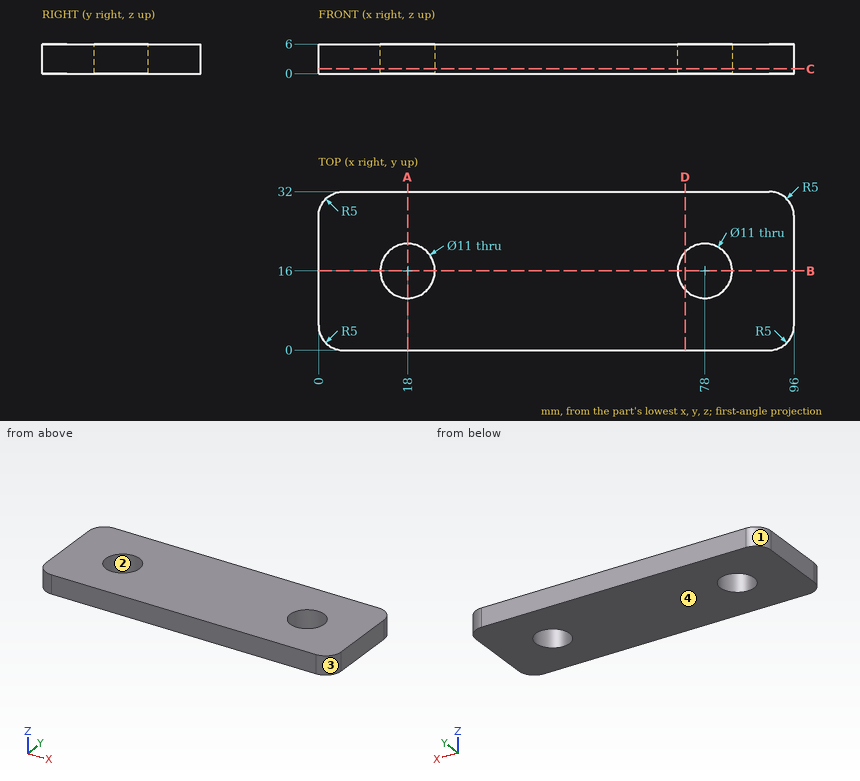
The drawing under review shows one solid part. Ordinate dimensions are in mm from its lowest x, y, z. Round coordinates to 2 decimals unless told otherwise and drop trailing zeros. Order: outer loops, then holes, each group sorted by start corner. A loop starts at its lowest first (then second) coordinate and runs counter-clockwise, first axis right, second up. Notation, with made-up numbers: (61, 83) -> (114, 83) arc R13 ccw to (114, 97) -> close; hole circle Ø1 at (21, -4). An arc over 180 degrees is marked (long way). Use a Markdown table: item, result.
Item 1: For pin 1 (10 mm diameter, centred on x = 78, y = 16, fed in from -Z), flat-tipped, find the tip position at first contact; note if it passes through.
Resolved:
| item | result |
|---|---|
| pin 1 | passes through |
Item 2: Take a section at C-C (z = 1). State the section outline as (x, y) points, plus the area to 3 significant figures.
Resolved:
| item | result |
|---|---|
| outline | (0, 5) arc R5 ccw to (5, 0) -> (91, 0) arc R5 ccw to (96, 5) -> (96, 27) arc R5 ccw to (91, 32) -> (5, 32) arc R5 ccw to (0, 27) -> close; hole circle Ø11 at (18, 16); hole circle Ø11 at (78, 16) |
| area | 2,860 mm² |
Item 3: For line 1 along Y through (x, z) = (78, 2); line 2 along X through (y, z) = (13, 4.55); line 3 along X through (y, z) = (15, 5.3), list the stretches that pass through material, from the lowest coordinate up. Write a range as [from, to].
Resolved:
| item | result |
|---|---|
| line 1 | y = [0, 10.5], [21.5, 32] |
| line 2 | x = [0, 13.39], [22.61, 73.39], [82.61, 96] |
| line 3 | x = [0, 12.59], [23.41, 72.59], [83.41, 96] |
Item 4: Draft analysis for pull direction X (two halves, no side actions). For the marked faces 1, 2, 3 and 4, state which applies: +X half, -X half, draft (parallel to the pull), parting line (faces both ways), or undercut.
Resolved:
| item | result |
|---|---|
| face 1 | -X half |
| face 2 | undercut |
| face 3 | +X half |
| face 4 | draft |
Item 5: Take a section at B-B (y = 16). State the section outline as (x, z) points, plus the area to 3 significant figures.
Resolved:
| item | result |
|---|---|
| outline | (0, 0) -> (12.5, 0) -> (12.5, 6) -> (0, 6) -> close; (23.5, 0) -> (72.5, 0) -> (72.5, 6) -> (23.5, 6) -> close; (83.5, 0) -> (96, 0) -> (96, 6) -> (83.5, 6) -> close |
| area | 444 mm² |
Item 6: Take a section at D-D (x = 74). State the section outline as (y, z) points.
Resolved:
| item | result |
|---|---|
| outline | (0, 0) -> (12.23, 0) -> (12.23, 6) -> (0, 6) -> close; (19.77, 0) -> (32, 0) -> (32, 6) -> (19.77, 6) -> close |
Item 7: Take a section at A-A (x = 18). State the section outline as (y, z) points.
Resolved:
| item | result |
|---|---|
| outline | (0, 0) -> (10.5, 0) -> (10.5, 6) -> (0, 6) -> close; (21.5, 0) -> (32, 0) -> (32, 6) -> (21.5, 6) -> close |
